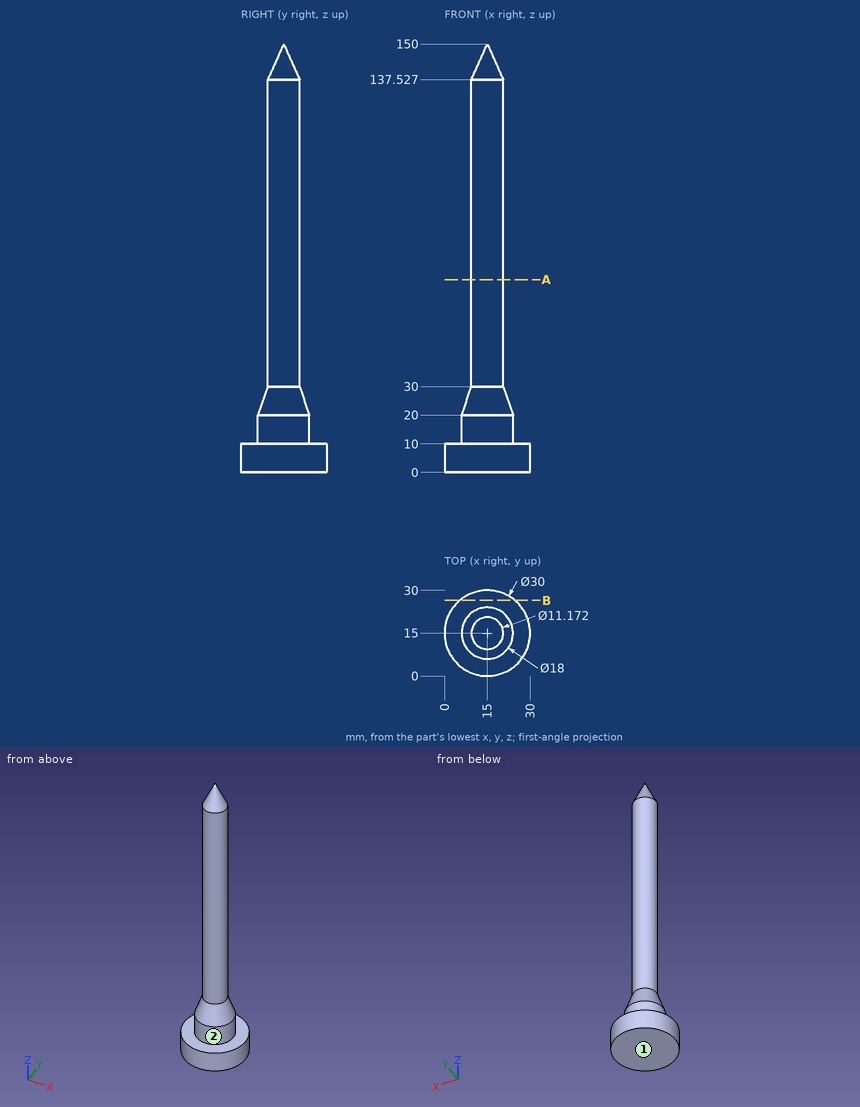
Design review of the part shown in the three views and the two pictorial views. Dimensions are in mm from the part's minimum x, y and z. A direction names the side the tool comes from. Coordinates: 2 decimals unless noted, no trailing zeros. Loops run counter-clockwise (first coordinate to the right, second up) from the corner with the lowest first, then second, coordinate; pieces in that order, holes last.
Q1. To check wall thickness, follow line 1 (Z direction, x = 4.25, y = 21.75); line 2 (Y direction, x = 20, z = 70); line 3 (Z direction, x = 13, y = 20) (1 decimal). State the ranges of each line that lie inside material, in increasing order.
Reported:
line 1: z = 0 to 10
line 2: y = 12.51 to 17.49
line 3: z = 0 to 138
Q2. We need section B-B on y = 26.5. State the section outline as (x, z) points.
Reported:
outline: (5.37, 0) - (24.63, 0) - (24.63, 10) - (5.37, 10) - close
Q3. For pin 1 (2 mm diameter, centred on x = 8, z = 88.5, fed in from -Y); pin 2 (10 mm diameter, centred on y = 22.5, z = 86, fed in from -X) (1 decimal); pin 3 (12 mm diameter, centred on x = 19, z = 110, fed in from -Y); pin 4 (10 mm diameter, centred on x = 17.5, z = 117.5, fed in from +Y), all flat-tipped, find the tip position at first contact; note any pin that passes through.
Reported:
pin 1: passes through
pin 2: stops at x = 10
pin 3: stops at y = 9.41
pin 4: stops at y = 20.59
Q4. We need section A-A on z = 67.5. State the section outline as (x, y) points.
Reported:
outline: circle Ø11.17 at (15, 15)
Q5. Tool access review of the marked faces 1 and 2: name each direction out of +Z, -Z, +X, -X, +Y, -Y from which nothing blocks a thin tool from reaching the whole face with its end or side.
Reported:
face 1: -Z, +X, -X, +Y, -Y
face 2: +Z
